```python
from build123d import *

# Parameters (mm, degrees)
ARCHED_PLATE_PROFILE_R      = 14
ARCHED_BASE_PLATE_DEPTH     = 5
SLOTTED_MOUNTING_FOOT_DEPTH = 10
CLEVIS_BLOCK_PROFILE_W      = 45
CLEVIS_BLOCK_PROFILE_H      = 40
CLEVIS_BLOCK_DEPTH          = 50
PLATE_EDGE_FILLET_RADIUS    = 20
PLATE_EDGE_FILLET_LENGTH    = 45
CLEVIS_PIN_HOLE_PROFILE_R   = 9
CLEVIS_PIN_HOLE_18_DEPTH    = 50
CLEVIS_SLOT_PROFILE_W       = 50
CLEVIS_SLOT_PROFILE_H       = 25
CLEVIS_SLOT_DEPTH           = 50


with BuildPart() as part:
    # Arched Plate Profile → Arched Base Plate (new, symmetric)
    with BuildSketch(Plane.XY):
        with BuildLine():
            Line((0, 0), (0, 17.91362622))
            ThreePointArc((0, 17.91362622), (20.718318638, 62.344203921), (68.071594305, 75.032475895))
            Line((68.071594305, 75.032475895), (119.569687178, 65.951972666))
            Line((119.569687178, 65.951972666), (112.623760072, 26.559662546))
            Line((112.623760072, 26.559662546), (93.472963553, 29.936464674))
            ThreePointArc((93.472963553, 29.936464674), (77.144247806, 25.561198476), (70, 10.240309613))
            Line((70, 10.240309613), (70, 0))
            Line((70, 0), (0, 0))
        make_face()
        with Locations((35, 24)):
            Circle(ARCHED_PLATE_PROFILE_R, mode=Mode.SUBTRACT)
    extrude(amount=ARCHED_BASE_PLATE_DEPTH, both=True)

    # Slotted Foot Profile → Slotted Mounting Foot (add)
    with BuildSketch(Plane(origin=(0, 0, 0), x_dir=(1, 0, 0), z_dir=(0, 1, 0))):
        with BuildLine():
            Line((0, -5), (70, -5))
            Line((70, -5), (70, -19))
            ThreePointArc((70, -19), (65.313708499, -30.313708499), (54, -35))
            Line((54, -35), (16, -35))
            ThreePointArc((16, -35), (4.686291501, -30.313708499), (0, -19))
            Line((0, -19), (0, -5))
        make_face()
        with BuildLine():
            Line((16, -12), (54, -12))
            ThreePointArc((54, -12), (62, -20), (54, -28))
            Line((54, -28), (16, -28))
            ThreePointArc((16, -28), (8, -20), (16, -12))
        make_face(mode=Mode.SUBTRACT)
    extrude(amount=SLOTTED_MOUNTING_FOOT_DEPTH)

    # Clevis Block Profile → Clevis Block (add)
    with BuildSketch(Plane(origin=(104.685768373, -18.45892546, 0), x_dir=(0, 0, -1), z_dir=(0.9848077530122075, -0.17364817766693413, 0))):
        with Locations((0, 65.713072291)):
            Rectangle(CLEVIS_BLOCK_PROFILE_W, CLEVIS_BLOCK_PROFILE_H)
    extrude(amount=CLEVIS_BLOCK_DEPTH)

    # Plate Edge Fillet: full round fillet: the end face becomes a half cylinder, R = half its width
    plate_edge_fillet_face = Plane((165.337111276, 37.573408722, 0), x_dir=(0, 0, -1), z_dir=(0.984807753012, -0.173648177667, 0))  # on the end face: x along it, z out of the body
    plate_edge_fillet_slab = plate_edge_fillet_face.offset(-PLATE_EDGE_FILLET_RADIUS / 2) * Box(PLATE_EDGE_FILLET_LENGTH, 2 * PLATE_EDGE_FILLET_RADIUS, PLATE_EDGE_FILLET_RADIUS, mode=Mode.PRIVATE)  # the body's end, R deep
    plate_edge_fillet_round = Plane((145.640956216, 41.046372275, 0), x_dir=(0.984807753012, -0.173648177667, 0), z_dir=(0, 0, -1)) * Cylinder(PLATE_EDGE_FILLET_RADIUS, PLATE_EDGE_FILLET_LENGTH, mode=Mode.PRIVATE)  # its axis R under the face
    add(plate_edge_fillet_slab - plate_edge_fillet_round, mode=Mode.SUBTRACT)

    # Clevis Pin Hole Profile → Clevis Pin Hole _18 (cut)
    with BuildSketch(Plane.XY.offset(22.5)):
        with Locations((145.640956215, 41.046372276)):
            Circle(CLEVIS_PIN_HOLE_PROFILE_R)
    extrude(amount=-CLEVIS_PIN_HOLE_18_DEPTH, mode=Mode.SUBTRACT)

    # Clevis Slot Profile → Clevis Slot (cut)
    with BuildSketch(Plane(origin=(14.883918806, 84.410898126, 0), x_dir=(0.9848077530122074, -0.17364817766693438, 0), z_dir=(0.17364817766693438, 0.9848077530122074, 0))):
        with Locations((141.300715091, 0)):
            Rectangle(CLEVIS_SLOT_PROFILE_W, CLEVIS_SLOT_PROFILE_H)
    extrude(amount=-CLEVIS_SLOT_DEPTH, mode=Mode.SUBTRACT)


solid = part.part
```
The listing builds one solid part. Answer for the finished solid, in the listing's coordinates (mm). A direction names the side the tool comes from. Round coordinates to 2 decimals unless told otherwise and drop trailing zeros. Write each loop counter-clockwise with the first axis right and the second up, starting at its lowest first coordinate (ties: lowest second). Pieces come first, ordered by that corner, then holes. Notation, with made-up numbers: (-16, 36) -> (-10, 36) arc R28 ccw to (-10, 68) -> close; hole circle Ø9 at (21, 14). An arc over 180 degrees is marked (long way). Answer as a JSON object with one key per item and string values. Group by question number.
Q1. Section B-B (z = 26) is taken. Write down the section's boundary in (x, y).
Q2. Section D-D (x = 152.5) is taken. Write down the section's boundary in (y, z), plus the area to 3 significant figures.
Q3. Section A-A (x = 38.5) is taken. Write down the section's boundary in (y, z), plus the area to 3 significant figures.
Q4. Which of the six approach directions +Z, -Z, +X, -X, +Y, -Y give full straight-line access (tool end or side, diameter ignored) to faces 5 (the face through (125.993, 44.795, 0.175)), 6 (the face through (70, 5, 7)), 7 (the face through (35, 10, 10))?
Q5. Determine the mould class of faces 1 (the face through (153.955, 37.599, 17.57)), 2 (the face through (136.66, 42.91, -12.5)), 3 (the face through (153.955, 37.599, -17.43)), 4 (the face through (20.178, 61.885, 0.07)) for opening direction Y: pulls with the +Y half, pulls with the -Y half, needs draft (parallel to the pull), parting line crosses it, or undercut.
Q6. Section C-C (y = 14) is taken. Write down the section's boundary in (x, z).
Q7. Each of these flat-tipped pins is pushed along its axis until it touches: pin 1 Ø11 at (x, y) = (30, 6.5) entering from -Z; pin 2 Ø5 at (x, y) = (145, 28.5) entering from +Z; pin 3 Ø15 at (x, z) = (19, 19) entering from +Y. Where does it stop, or does it pass through?
Q8. Straight lines are drawn through the part: line 1 along Z through (x, y) = (148, 53); line 2 along Y through (x, z) = (11.5, 31.5); line 3 along Z through (x, y) = (65, 11.5). For each, find the intervals that lie inside material, in ascending order.
Check values:
{
 "1": {"outline": "(1.61, 0) -> (10.71, 0) -> (10.71, 10) -> (1.61, 10) -> close; (59.29, 0) -> (68.39, 0) -> (68.39, 10) -> (59.29, 10) -> close"},
 "2": {"outline": "(22.26, -22.5) -> (35.22, -22.5) -> (35.22, -12.5) -> (22.26, -12.5) -> close; (22.26, 12.5) -> (35.22, 12.5) -> (35.22, 22.5) -> (22.26, 22.5) -> close; (46.87, -22.5) -> (59.83, -22.5) -> (59.83, -12.5) -> (46.87, -12.5) -> close; (46.87, 12.5) -> (59.83, 12.5) -> (59.83, 22.5) -> (46.87, 22.5) -> close", "area": "518 mm^2"},
 "3": {"outline": "(0, -5) -> (10.44, -5) -> (10.44, 5) -> (10, 5) -> (10, 12) -> (0, 12) -> close; (0, 28) -> (10, 28) -> (10, 35) -> (0, 35) -> close; (37.56, -5) -> (72.54, -5) -> (72.54, 5) -> (37.56, 5) -> close", "area": "594 mm^2"},
 "4": {"face 5": "+X, -Y", "face 6": "+Z, -Z, +X, -Y", "face 7": "+Z, +X, -X, +Y"},
 "5": {"face 1": "undercut", "face 2": "needs draft", "face 3": "undercut", "face 4": "pulls with the +Y half"},
 "6": {"outline": "(0, -5) -> (25.2, -5) -> (25.2, 5) -> (0, 5) -> close; (44.8, -5) -> (70.36, -5) -> (70.36, 5) -> (44.8, 5) -> close"},
 "7": {"pin 1": "z = -5", "pin 2": "z = 22.5", "pin 3": "y = 10"},
 "8": {"line 1": "-22.5 to -12.5, 12.5 to 22.5", "line 2": "0 to 10", "line 3": "-5 to 5"}
}
